CAD build for the part. Positions are in the model's coordinates, mm. Face numbers are marked on the shaded views. Give positions to 0.01 mm unless a question says otherwise; leave off trailing zeros. Write each loop counter-clockwise with the first axis right and the second up, starting at its lowest first coordinate (ties: lowest second). Pieces come first, ordered by that corner, then holes. Notation, with made-up numbers: M -14.75,37 L -5.75,37 A27 ccw -5.75,56 Z; hole C -27.75,51 d8. An arc over 180 degrees is marked long. One line per question, with ' | ' between items. Start each with the question number.
1. Cut at C-C, the plane z = 7.75. Write the cut outline in (x, y), then the cut area to 3 significant figures.
2. Cut at A-A, the plane y = 0.8. Write the cut outline in (x, z).
3. Flat gauge pin, fed straight in: pin 1 (2 mm diameter, centred on x = -32, y = 22, fed in from -Z). Where does the tip first touch, or does it go through?
4. Pull direction Y, two halves, no side cores. Call the marked faces 1, 2 and 3: released by +Y, released by -Y, zero draft, split by the parting line, or undercut.
5. Wall check: L1, parallel to Y at x = 19.1, z = 7.5. Give the ranges that are in metal, low to high.
6. Cut at B-B, the plane x = -23.9. Write the cut outline in (y, z).
```python
from build123d import *

# Parameters (mm, degrees)
EXTRUDE_1_DEPTH             = 10
HOLE_WIZARD_14_0_14_1_D     = 14
HOLE_WIZARD_14_0_14_1_DEPTH = 19.793975667
HOLE_WIZARD_14_0_14_1_TIP   = 4.206024333


with BuildPart() as part:
    # 草图1 → 凸台-拉伸1 (new body)
    with BuildSketch(Plane.XY):
        with BuildLine():
            Line((-42.5, 40), (37.5, 40))
            ThreePointArc((37.5, 40), (41.035533906, 38.535533906), (42.5, 35))
            Line((42.5, 35), (42.5, -35))
            ThreePointArc((42.5, -35), (41.035533906, -38.535533906), (37.5, -40))
            Line((37.5, -40), (-42.5, -40))
            Line((-42.5, -40), (-42.5, 40))
        make_face()
    extrude(amount=EXTRUDE_1_DEPTH)

    # Ø14.0 (14) 直径孔1
    with Locations(Plane.XY.offset(10)):
        with Locations((19.1, 0.8), (-23.9, 0.8)):
            Hole(HOLE_WIZARD_14_0_14_1_D / 2, depth=HOLE_WIZARD_14_0_14_1_DEPTH)
            with Locations((0, 0, -(HOLE_WIZARD_14_0_14_1_DEPTH + HOLE_WIZARD_14_0_14_1_TIP / 2))):  # 118° drill point
                Cone(0, HOLE_WIZARD_14_0_14_1_D / 2, HOLE_WIZARD_14_0_14_1_TIP, mode=Mode.SUBTRACT)


solid = part.part
```
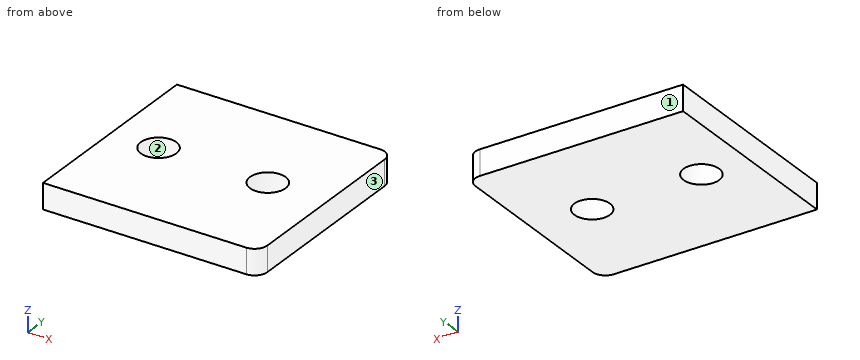
Here are the results:
1) outline: M -42.5,-40 L 37.5,-40 A5 ccw 42.5,-35 L 42.5,35 A5 ccw 37.5,40 L -42.5,40 Z; hole C -23.9,0.8 d14; hole C 19.1,0.8 d14 | area: 6,480 mm^2
2) outline: M -42.5,0 L -30.9,0 L -30.9,10 L -42.5,10 Z; M -16.9,0 L 12.1,0 L 12.1,10 L -16.9,10 Z; M 26.1,0 L 42.5,0 L 42.5,10 L 26.1,10 Z
3) pin 1: z = 0
4) face 1: released by +Y | face 2: undercut | face 3: zero draft
5) L1: -40 to -6.2, 7.8 to 40
6) outline: M -40,0 L -6.2,0 L -6.2,10 L -40,10 Z; M 7.8,0 L 40,0 L 40,10 L 7.8,10 Z
